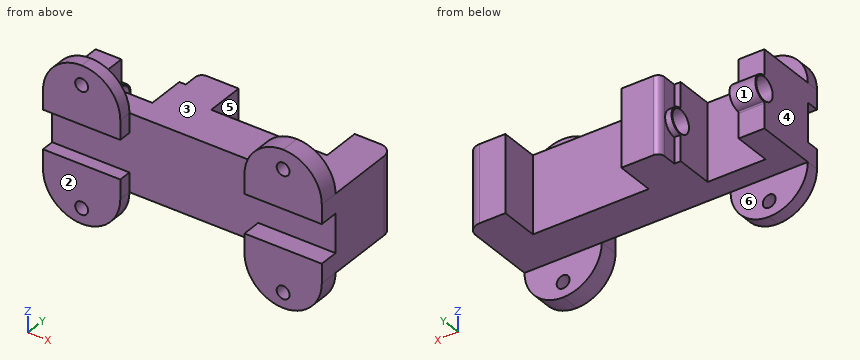
from build123d import *

# Parameters (mm, degrees)
BASE_PLATE_DEPTH           = 15
BODY_BLOCK_SKETCH_W        = 200
BODY_BLOCK_SKETCH_H        = 60
BODY_BLOCK_DEPTH           = 48
FIXED_JAW_SKETCH_W         = 60
FIXED_JAW_SKETCH_H         = 63
FIXED_JAW_DEPTH            = 20
GUIDE_CHANNEL_SKETCH_W     = 60
GUIDE_CHANNEL_SKETCH_H     = 60
GUIDE_CHANNEL_CUT_DEPTH    = 30
CHANNEL_END_CUT_SKETCH_W   = 30
CHANNEL_END_CUT_SKETCH_H   = 60
CHANNEL_END_CUT_DEPTH      = 30
JAW_SLOT_SKETCH_W          = 50
JAW_SLOT_SKETCH_H          = 60
JAW_SLOT_CUT_DEPTH         = 45
SLOT_RAIL_SKETCH_R         = 10
SLOT_RAIL_DEPTH            = 5
SCREW_BORE_SKETCH_R        = 9
SCREW_BORE_DEPTH           = 79
SCREW_POCKET_CUT_DEPTH     = 40
SCREW_BOSS_SKETCH_R        = 10
SCREW_BOSS_SKETCH_R_2      = 9
SCREW_BOSS_DEPTH           = 20
FIXED_JAW_FILLET_R10_R     = 10
JAW_SLOT_FILLET_R5_R       = 5
SCREW_BOSS_FILLET_R1_A_R   = 1
SCREW_BOSS_FILLET_R1_B_R   = 1
MOUNTING_FLANGE_SKETCH_W   = 60
MOUNTING_FLANGE_SKETCH_H   = 10
MOUNTING_FLANGE_DEPTH      = 30
FLANGE_RECESS_CUT_DEPTH    = 15
MOUNTING_LUG_SKETCH_W      = 60
MOUNTING_LUG_SKETCH_H      = 10
MOUNTING_LUG_DEPTH         = 15
REAR_JAW_BLOCK_SKETCH_W    = 60
REAR_JAW_BLOCK_SKETCH_H    = 15
REAR_JAW_BLOCK_DEPTH       = 30
REAR_JAW_CHANNEL_CUT_DEPTH = 30
REAR_JAW_NOTCH_CUT_DEPTH   = 30
REAR_LUG_SKETCH_W          = 60
REAR_LUG_SKETCH_H          = 15
REAR_LUG_DEPTH             = 15
LUG_CLEARANCE_CUT_SKETCH_R = 5
LUG_CLEARANCE_CUT_DEPTH    = 15


with BuildPart() as part:
    # Base Plate Sketch → Base Plate (new body)
    with BuildSketch(Plane(origin=(0, 0, 0), x_dir=(1, 0, 0), z_dir=(0, 1, 0))):
        Polygon((0, 0), (100, 0), (100, 60), (-100, 60), (-100, 0), align=None)
    extrude(amount=BASE_PLATE_DEPTH)

    # Body Block Sketch → Body Block (add)
    with BuildSketch(Plane(origin=(0, 15, 0), x_dir=(1, 0, 0), z_dir=(0, 1, 0))):
        with Locations((0, 30)):
            Rectangle(BODY_BLOCK_SKETCH_W, BODY_BLOCK_SKETCH_H)
    extrude(amount=BODY_BLOCK_DEPTH)

    # Fixed Jaw Sketch → Fixed Jaw (add)
    with BuildSketch(Plane(origin=(100, 0, 0), x_dir=(0, 0, -1), z_dir=(1, 0, 0))):
        with Locations((30, 31.5)):
            Rectangle(FIXED_JAW_SKETCH_W, FIXED_JAW_SKETCH_H)
    extrude(amount=FIXED_JAW_DEPTH)

    # Guide Channel Sketch → Guide Channel Cut (cut)
    with BuildSketch(Plane(origin=(0, 63, 0), x_dir=(1, 0, 0), z_dir=(0, 1, 0))):
        with Locations((60, 30)):
            Rectangle(GUIDE_CHANNEL_SKETCH_W, GUIDE_CHANNEL_SKETCH_H)
    extrude(amount=-GUIDE_CHANNEL_CUT_DEPTH, mode=Mode.SUBTRACT)

    # Channel End Cut Sketch → Channel End Cut (cut)
    with BuildSketch(Plane(origin=(0, 63, 0), x_dir=(1, 0, 0), z_dir=(0, 1, 0))):
        with Locations((15, 30)):
            Rectangle(CHANNEL_END_CUT_SKETCH_W, CHANNEL_END_CUT_SKETCH_H)
    extrude(amount=-CHANNEL_END_CUT_DEPTH, mode=Mode.SUBTRACT)

    # Jaw Slot Sketch → Jaw Slot Cut (cut)
    with BuildSketch(Plane(origin=(0, 63, 0), x_dir=(1, 0, 0), z_dir=(0, 1, 0))):
        with Locations((-55, 30)):
            Rectangle(JAW_SLOT_SKETCH_W, JAW_SLOT_SKETCH_H)
    extrude(amount=-JAW_SLOT_CUT_DEPTH, mode=Mode.SUBTRACT)

    # Slot Rail Sketch → Slot Rail (add)
    with BuildSketch(Plane.ZY.offset(30)):
        with Locations((-30, 47.357372748)):
            Circle(SLOT_RAIL_SKETCH_R)
        with BuildLine():
            Line((0, 18), (0, 47.357372748))
            Line((0, 47.357372748), (-20, 47.357372748))
            ThreePointArc((-20, 47.357372748), (-30, 37.357372748), (-40, 47.357372748))
            Line((-40, 47.357372748), (-60, 47.357372748))
            Line((-60, 47.357372748), (-60, 18))
            Line((-60, 18), (0, 18))
        make_face()
    extrude(amount=SLOT_RAIL_DEPTH)

    # Screw Bore Sketch → Screw Bore (cut, symmetric)
    with BuildSketch(Plane.ZY.offset(35)):
        with Locations((-30, 47.357372748)):
            Circle(SCREW_BORE_SKETCH_R)
    extrude(amount=SCREW_BORE_DEPTH, both=True, mode=Mode.SUBTRACT)

    # Screw Pocket Sketch → Screw Pocket Cut (cut)
    with BuildSketch(Plane.ZY.offset(100)):
        with BuildLine():
            ThreePointArc((-39, 47.357372748), (-30, 56.357372748), (-21, 47.357372748))
            Line((-21, 47.357372748), (0, 47.357372748))
            Line((0, 47.357372748), (0, 63))
            Line((0, 63), (-60, 63))
            Line((-60, 63), (-60, 47.357372748))
            Line((-60, 47.357372748), (-39, 47.357372748))
        make_face()
    extrude(amount=-SCREW_POCKET_CUT_DEPTH, mode=Mode.SUBTRACT)

    # Screw Boss Sketch → Screw Boss (add)
    with BuildSketch(Plane.ZY.offset(100)):
        with Locations((-30, 47.357372748)):
            Circle(SCREW_BOSS_SKETCH_R)
        with Locations(Location((-30, 47.357372748, 0), (0, 0, 180))):
            Circle(SCREW_BOSS_SKETCH_R_2, mode=Mode.SUBTRACT)
    extrude(amount=-SCREW_BOSS_DEPTH)

    # Fixed Jaw Fillet R10
    fixed_jaw_fillet_r10_edges = [part.edges().sort_by_distance(p)[0] for p in [
        (120, 63, -30),
    ]]
    fillet(fixed_jaw_fillet_r10_edges, radius=FIXED_JAW_FILLET_R10_R)

    # Jaw Slot Fillet R5
    jaw_slot_fillet_r5_edges = [part.edges().sort_by_distance(p)[0] for p in [
        (-30, 63, -30),
    ]]
    fillet(jaw_slot_fillet_r5_edges, radius=JAW_SLOT_FILLET_R5_R)

    # Screw Boss Fillet R1 A
    screw_boss_fillet_r1_a_edges = [part.edges().sort_by_distance(p)[0] for p in [
        (-90, 47.357372748, -20),
    ]]
    fillet(screw_boss_fillet_r1_a_edges, radius=SCREW_BOSS_FILLET_R1_A_R)

    # Screw Boss Fillet R1 B
    screw_boss_fillet_r1_b_edges = [part.edges().sort_by_distance(p)[0] for p in [
        (-90, 47.357372748, -40),
    ]]
    fillet(screw_boss_fillet_r1_b_edges, radius=SCREW_BOSS_FILLET_R1_B_R)



with BuildPart() as body_2:
    # Mounting Flange Sketch → Mounting Flange (new body)
    with BuildSketch(Plane.XY):
        with Locations((-70, -5)):
            Rectangle(MOUNTING_FLANGE_SKETCH_W, MOUNTING_FLANGE_SKETCH_H)
    extrude(amount=MOUNTING_FLANGE_DEPTH)

    # Flange Recess Sketch → Flange Recess Cut (cut)
    with BuildSketch(Plane(origin=(0, 0, 0), x_dir=(1, 0, 0), z_dir=(0, 1, 0))):
        with BuildLine():
            Line((-40, -30), (-40, 0))
            ThreePointArc((-40, 0), (-48.786796564, -21.213203436), (-70, -30))
            Line((-70, -30), (-40, -30))
        make_face()
        with BuildLine():
            Line((-100, -30), (-70, -30))
            ThreePointArc((-70, -30), (-91.213203436, -21.213203436), (-100, 0))
            Line((-100, 0), (-100, -30))
        make_face()
    extrude(amount=-FLANGE_RECESS_CUT_DEPTH, mode=Mode.SUBTRACT)


with BuildPart() as part_1:
    add(part.part)

    add(body_2.part)  # Mounting Lug merges body 2
    # Mounting Lug Sketch → Mounting Lug (add)
    with BuildSketch(Plane(origin=(0, 0, 0), x_dir=(-1, 0, 0), z_dir=(0, 0, -1))):
        with Locations((70, -5)):
            Rectangle(MOUNTING_LUG_SKETCH_W, MOUNTING_LUG_SKETCH_H)
    extrude(amount=MOUNTING_LUG_DEPTH)

    # Mounting Lug Mirror: part across plane


with BuildPart() as part_2:
    add(part_1.part)
    add(part_1.part.mirror(Plane.XY.offset(-30)))



with BuildPart() as body_2_2:
    # Rear Jaw Block Sketch → Rear Jaw Block (new body)
    with BuildSketch(Plane.XY):
        with Locations((90, -7.5)):
            Rectangle(REAR_JAW_BLOCK_SKETCH_W, REAR_JAW_BLOCK_SKETCH_H)
    extrude(amount=REAR_JAW_BLOCK_DEPTH)

    # Rear Jaw Channel Sketch → Rear Jaw Channel Cut (cut)
    with BuildSketch(Plane(origin=(0, 0, 0), x_dir=(1, 0, 0), z_dir=(0, 1, 0))):
        with BuildLine():
            ThreePointArc((90, -30), (68.786796564, -21.213203436), (60, 0))
            Line((60, 0), (60, -30))
            Line((60, -30), (90, -30))
        make_face()
    extrude(amount=-REAR_JAW_CHANNEL_CUT_DEPTH, mode=Mode.SUBTRACT)

    # Rear Jaw Notch Sketch → Rear Jaw Notch Cut (cut)
    with BuildSketch(Plane(origin=(0, 0, 0), x_dir=(1, 0, 0), z_dir=(0, 1, 0))):
        with BuildLine():
            Line((120, -30), (120, 0))
            ThreePointArc((120, 0), (111.213203436, -21.213203436), (90, -30))
            Line((90, -30), (120, -30))
        make_face()
    extrude(amount=-REAR_JAW_NOTCH_CUT_DEPTH, mode=Mode.SUBTRACT)


with BuildPart() as part_3:
    add(part_2.part)

    add(body_2_2.part)  # Rear Lug merges body 2 2
    # Rear Lug Sketch → Rear Lug (add)
    with BuildSketch(Plane(origin=(0, 0, 0), x_dir=(-1, 0, 0), z_dir=(0, 0, -1))):
        with Locations((-90, -7.5)):
            Rectangle(REAR_LUG_SKETCH_W, REAR_LUG_SKETCH_H)
    extrude(amount=REAR_LUG_DEPTH)

    # Rear Lug Mirror: part across plane


with BuildPart() as part_4:
    add(part_3.part)
    add(part_3.part.mirror(Plane.XY.offset(-30)))

    # Lug Clearance Cut Sketch → Lug Clearance Cut (cut)
    with BuildSketch(Plane(origin=(0, 0, 0), x_dir=(1, 0, 0), z_dir=(0, 1, 0))):
        with Locations(Location((-70, -15.138677931, 0), (0, 0, 270))):
            Circle(LUG_CLEARANCE_CUT_SKETCH_R)
        with Locations(Location((90, -15.138677931, 0), (0, 0, 270))):
            Circle(LUG_CLEARANCE_CUT_SKETCH_R)
        with Locations(Location((-70, 78.223643899, 0), (0, 0, 270))):
            Circle(LUG_CLEARANCE_CUT_SKETCH_R)
        with Locations(Location((90, 78.223643899, 0), (0, 0, 270))):
            Circle(LUG_CLEARANCE_CUT_SKETCH_R)
    extrude(amount=-LUG_CLEARANCE_CUT_DEPTH, mode=Mode.SUBTRACT)


solid = part_4.part
The listing builds one solid part. Answer for the finished solid, in the listing's coordinates (mm). Face numbers are marked on the shaded views. A direction names the side the tool comes from. Give positions to 0.01 mm unless a question says otherwise; leave off trailing zeros. Write each loop counter-clockwise with the first axis right and the second up, starting at its lowest first coordinate (ties: lowest second). Pieces come first, ordered by that corner, then holes.
Item 1: Section C-C, the plane z = 5 is taken. Write down the section's boundary in (x, y), plus the area to 3 significant figures.
Item 2: Section B-B, the plane y = 28.5 is taken. Write down the section's boundary in (x, z), plus the area to 3 significant figures.
Item 3: Determine the mould class of the marked faces 4, 5 and 6 for opening direction X: released by +X, released by -X, zero draft, split by the parting line, or undercut.
Item 4: Section A-A, the plane z = -30 is taken. Write down the section's boundary in (x, y), plus the area to 3 significant figures.
Item 5: Section D-D, the plane x = 65 is taken. Write down the section's boundary in (y, z).
Item 6: Which of the six approach directions +Z, -Z, +X, -X, +Y, -Y give full straight-line access (tool end or side, diameter ignored) to the marked faces 1, 2 and 3?
Item 7: Flat-ended cylindrical pins translate along their axes: P1, Ø15, axis at x = 103.5, z = 20.5, coming from the +Y side; P2, Ø5, axis at x = -84, y = -7, coming from the +Z side; P3, Ø3, axis at x = -83, y = -3, coming from the -Z side. Find the tip coordinate at first contact, or state that the pin passes through.
Item 8: Find the intervals of material crossed by line 1 along X through (y, z) = (35, -15); line 2 along Y through (x, z) = (-95.5, -30); line 3 along Y through (x, z) = (101, -37), in increasing order.
Completed:
1. outline: (-99.58, -10) - (-40.42, -10) - (-40.42, 0) - (-99.58, 0) - close; (60.42, -15) - (119.58, -15) - (119.58, 0) - (60.42, 0) - close
1. area: 1,480 mm2
2. outline: (-100, -60) - (-80, -60) - (-80, 0) - (-100, 0) - close; (-35, -60) - (120, -60) - (120, 0) - (-35, 0) - close
2. area: 10,500 mm2
3. face 4: released by -X
3. face 5: undercut
3. face 6: zero draft
4. outline: (-100, 0) - (120, 0) - (120, 53) arc R10 ccw to (110, 63) - (90, 63) - (90, 33) - (0, 33) - (0, 38.36) - (-35, 38.36) - (-35, 18) - (-80, 18) - (-80, 38.36) - (-100, 38.36) - close; (-100, 56.36) - (-80, 56.36) - (-80, 57.36) - (-100, 57.36) - close; (-35, 56.36) - (0, 56.36) - (0, 63) - (-25, 63) arc R5 ccw to (-30, 58) - (-30, 57.36) - (-35, 57.36) - close
4. area: 7,980 mm2
5. outline: (-15, -76.58) - (0, -76.58) - (0, -60) - (33, -60) - (33, 0) - (0, 0) - (0, 16.58) - (-15, 16.58) - (-15, -15) - (0, -15) - (0, -45) - (-15, -45) - close
6. face 1: -X, +Y
6. face 2: +Z, -Z, -X, -Y
6. face 3: +Z, +X, -X, +Y
7. P1: stops at y = 0
7. P2: stops at z = 27.71
7. P3: stops at z = -87.71
8. line 1: x = -100 to -80, -35 to 0, 90 to 120
8. line 2: y = 0 to 38.36, 56.36 to 57.36
8. line 3: y = 0 to 63
